```python
from build123d import *

# Parameters (mm, degrees)
SKETCH_1_W                = 80
SKETCH_1_H                = 180
EXTRUDE_1_DEPTH           = 15
CHAMFER_1_SIZE            = 3
HOLE_WIZARD_M4_1_D        = 3.3
HOLE_WIZARD_M4_1_DEPTH    = 20
HOLE_WIZARD_M4_1_TIP      = 0.991420021
HOLE_WIZARD_1_D           = 5.5
HOLE_WIZARD_1_DEPTH       = 20
HOLE_WIZARD_1_CBORE_D     = 10
HOLE_WIZARD_1_CBORE_DEPTH = 5.7
HOLE_WIZARD_1_TIP         = 1.652366702
HOLE_WIZARD_2_D           = 5.5
HOLE_WIZARD_2_DEPTH       = 15
HOLE_WIZARD_2_CBORE_D     = 10
HOLE_WIZARD_2_CBORE_DEPTH = 5.7
HOLE_WIZARD_2_TIP         = 1.652366702


with BuildPart() as part:
    # 草图1 → 凸台-拉伸1 (new body)
    with BuildSketch(Plane(origin=(0, 0, 0), x_dir=(1, 0, 0), z_dir=(0, 1, 0))):
        Rectangle(SKETCH_1_W, SKETCH_1_H)
    extrude(amount=EXTRUDE_1_DEPTH)

    # 倒角1
    chamfer_1_edges = [part.edges().sort_by_distance(p)[0] for p in [
        (40, 7.5, 90),
        (-40, 7.5, 90),
        (-40, 7.5, -90),
        (40, 7.5, -90),
    ]]
    chamfer(chamfer_1_edges, length=CHAMFER_1_SIZE)

    # M4 螺纹孔1
    with Locations(Plane(origin=(0, 15, 0), x_dir=(1, 0, 0), z_dir=(0, 1, 0))):
        with Locations((0, 60), (0, 5)):
            Hole(HOLE_WIZARD_M4_1_D / 2, depth=HOLE_WIZARD_M4_1_DEPTH)
            with Locations((0, 0, -(HOLE_WIZARD_M4_1_DEPTH + HOLE_WIZARD_M4_1_TIP / 2))):  # 118° drill point
                Cone(0, HOLE_WIZARD_M4_1_D / 2, HOLE_WIZARD_M4_1_TIP, mode=Mode.SUBTRACT)

    # 打孔尺寸(%根据)内六角圆柱头螺钉的类型1
    with Locations(Plane(origin=(0, 15, 0), x_dir=(1, 0, 0), z_dir=(0, 1, 0))):
        with Locations((-30, -27.5), (0, -27.5), (30, -27.5)):
            CounterBoreHole(HOLE_WIZARD_1_D / 2, HOLE_WIZARD_1_CBORE_D / 2, HOLE_WIZARD_1_CBORE_DEPTH, depth=HOLE_WIZARD_1_DEPTH)
            with Locations((0, 0, -(HOLE_WIZARD_1_DEPTH + HOLE_WIZARD_1_TIP / 2))):  # 118° drill point
                Cone(0, HOLE_WIZARD_1_D / 2, HOLE_WIZARD_1_TIP, mode=Mode.SUBTRACT)

    # 打孔尺寸(%根据)内六角圆柱头螺钉的类型2
    with Locations(Plane(origin=(0, 15, 0), x_dir=(1, 0, 0), z_dir=(0, 1, 0))):
        with Locations((-30, -75), (0, -75), (30, -75)):
            CounterBoreHole(HOLE_WIZARD_2_D / 2, HOLE_WIZARD_2_CBORE_D / 2, HOLE_WIZARD_2_CBORE_DEPTH, depth=HOLE_WIZARD_2_DEPTH)
            with Locations((0, 0, -(HOLE_WIZARD_2_DEPTH + HOLE_WIZARD_2_TIP / 2))):  # 118° drill point
                Cone(0, HOLE_WIZARD_2_D / 2, HOLE_WIZARD_2_TIP, mode=Mode.SUBTRACT)


solid = part.part
```
Design review of the part built by this model. Coordinates are the model's own, in mm. A direction names the side the tool comes from. Round coordinates to 2 decimals unless told otherwise and drop trailing zeros. Write each loop counter-clockwise with the first axis right and the second up, starting at its lowest first coordinate (ties: lowest second). Pieces come first, ordered by that corner, then holes. Notation, with made-up numbers: (44, 63.5) -> (58, 63.5) arc R19 ccw to (58, 76.5) -> close; hole circle Ø1 at (61, 20.25). An arc over 180 degrees is marked (long way). Write item = value, one per line. Start each with the question number.
1) Take a section at A-A, the plane z = 75. State the section outline as (x, y) points, plus the area to 3 significant figures.
2) Mouldability with a two-part tool opening along Z and no side actions: class faces 3 (the face through (-31.08, 12.19, 79.88)), 4 (the face through (39, 7, 88)), 5 (the face through (-1, 15, -1)) as +Z half, -Z half, draft (parallel to the pull), parting line (faces both ways), or undercut.
3) Take a section at B-B, the plane x = 0. State the section outline as (y, z) points, plus the area to 3 significant figures.
4) Wall thickness on probe 1 along Z at (x, y) = (0, 2); probe 2 along Z at (x, y) = (0, 10.5); probe 3 along Z at (x, y) = (-30, 5.5): over which ranges is each line inside the solid? List them lowest first. Write a range as from..to.
5) Tool access review of faces 1 (the face through (-1.08, 12.19, 32.38)), 2 (the face through (-40, 7, 1)): name each direction out of +Z, -Z, +X, -X, +Y, -Y from which nothing blocks a thin tool from reaching the whole face with its end or side.
6) Take a section at D-D, the plane z = -5. State the section outline as (x, y) points.
7) Take a section at C-C, the plane x = 30. State the section outline as (y, z) points, plus the area to 3 significant figures.
8) Clearance check with a flat-ended pin moving along its axis: pin 1 (5 mm diameter, centred on x = 29, z = 76, fed in from +Y). State where the tip first meets the part, or that it passes through.
Results list:
q1.outline = (-40, 0) -> (-32.75, 0) -> (-32.75, 9.3) -> (-35, 9.3) -> (-35, 15) -> (-40, 15) -> close; (-27.25, 0) -> (-2.75, 0) -> (-2.75, 9.3) -> (-5, 9.3) -> (-5, 15) -> (-25, 15) -> (-25, 9.3) -> (-27.25, 9.3) -> close; (2.75, 0) -> (27.25, 0) -> (27.25, 9.3) -> (25, 9.3) -> (25, 15) -> (5, 15) -> (5, 9.3) -> (2.75, 9.3) -> close; (32.75, 0) -> (40, 0) -> (40, 15) -> (35, 15) -> (35, 9.3) -> (32.75, 9.3) -> close
q1.area = 876 mm²
q2.face_3 = undercut
q2.face_4 = +Z half
q2.face_5 = draft
q3.outline = (0, -90) -> (15, -90) -> (15, -61.65) -> (0, -61.65) -> close; (0, -58.35) -> (15, -58.35) -> (15, -6.65) -> (0, -6.65) -> close; (0, -3.35) -> (15, -3.35) -> (15, 22.5) -> (9.3, 22.5) -> (9.3, 24.75) -> (0, 24.75) -> close; (0, 30.25) -> (9.3, 30.25) -> (9.3, 32.5) -> (15, 32.5) -> (15, 70) -> (9.3, 70) -> (9.3, 72.25) -> (0, 72.25) -> close; (0, 77.75) -> (9.3, 77.75) -> (9.3, 80) -> (15, 80) -> (15, 90) -> (0, 90) -> close
q3.area = 2,380 mm²
q4.probe_1 = -90..-61.65, -58.35..-6.65, -3.35..24.75, 30.25..72.25, 77.75..90
q4.probe_2 = -90..-61.65, -58.35..-6.65, -3.35..22.5, 32.5..70, 80..90
q4.probe_3 = -90..24.75, 30.25..72.25, 77.75..90
q5.face_1 = +Y
q5.face_2 = +Z, -Z, -X, +Y, -Y
q6.outline = (-40, 0) -> (-1.65, 0) -> (-1.65, 15) -> (-40, 15) -> close; (1.65, 0) -> (40, 0) -> (40, 15) -> (1.65, 15) -> close
q7.outline = (0, -90) -> (15, -90) -> (15, 22.5) -> (9.3, 22.5) -> (9.3, 24.75) -> (0, 24.75) -> close; (0, 30.25) -> (9.3, 30.25) -> (9.3, 32.5) -> (15, 32.5) -> (15, 70) -> (9.3, 70) -> (9.3, 72.25) -> (0, 72.25) -> close; (0, 77.75) -> (9.3, 77.75) -> (9.3, 80) -> (15, 80) -> (15, 90) -> (0, 90) -> close
q7.area = 2,480 mm²
q8.pin_1 = 9.3
